from build123d import *

# Parameters (mm, degrees)
BASE_BODY_DEPTH           = 23
FORK_SLOT_19X15_REACH     = 72.915
FORK_SLOT_SKETCH_W        = 19
FORK_SLOT_SKETCH_H        = 15
CHANNEL_CUT_SKETCH_W      = 19
CHANNEL_CUT_SKETCH_H      = 40
THIN_CHANNEL_CUT_19_DEPTH = 15
LUG_SKETCH_R              = 10
LUG_WITH_BORE_DEPTH       = 10
SUPPORT_RIB_REACH         = 82.206
SUPPORT_RIB_SKETCH_WALL_W = 191.480853336
SUPPORT_RIB_SKETCH_WALL_H = 46


with BuildPart() as part:
    # Base Profile Sketch → Base Body (new, symmetric)
    with BuildSketch(Plane(origin=(0, 0, 0), x_dir=(0, 0, -1), z_dir=(1, 0, 0))):
        Polygon((-60, 0), (40, 0), (40, -15), (10, -15), (10, -30), (-30, -30), (-30, -15), (-60, -15), align=None)
    extrude(amount=BASE_BODY_DEPTH, both=True)

    # Fork Slot Sketch → Fork Slot 19x15 (cut, up to next)
    with BuildSketch(Plane(origin=(0, 0, 0), x_dir=(1, 0, 0), z_dir=(0, 1, 0)), mode=Mode.PRIVATE) as fork_slot_19x15_sk1:
        with Locations((0, -52.5)):
            Rectangle(FORK_SLOT_SKETCH_W, FORK_SLOT_SKETCH_H)
    fork_slot_19x15_tool1 = extrude(fork_slot_19x15_sk1.sketch, amount=-FORK_SLOT_19X15_REACH, mode=Mode.PRIVATE) & part.part
    add(fork_slot_19x15_tool1.solids().sort_by_distance((0, 0, 52.5))[0], mode=Mode.SUBTRACT)

    # Channel Cut Sketch → Thin Channel Cut 19 (cut)
    with BuildSketch(Plane.XZ.offset(30)):
        with Locations((0, 10)):
            Rectangle(CHANNEL_CUT_SKETCH_W, CHANNEL_CUT_SKETCH_H)
    extrude(amount=-THIN_CHANNEL_CUT_19_DEPTH, mode=Mode.SUBTRACT)

    # Lug Sketch → Lug with Bore (add)
    with BuildSketch(Plane.XY):
        with BuildLine():
            Line((23, 25), (23, 0))
            Line((23, 0), (-23, 0))
            Line((-23, 0), (-23, 25))
            ThreePointArc((-23, 25), (0, 48), (23, 25))
        make_face()
        with Locations((0, 25)):
            Circle(LUG_SKETCH_R, mode=Mode.SUBTRACT)
    extrude(amount=LUG_WITH_BORE_DEPTH)

    # Support Rib Sketch wall → Support Rib (add, up to next)
    with BuildSketch(Plane(origin=(0, 6.5, 23), x_dir=(0, -0.4472135955, 0.894427191), z_dir=(0, -0.894427191, -0.4472135955)), mode=Mode.PRIVATE) as support_rib_sk1:
        Rectangle(SUPPORT_RIB_SKETCH_WALL_W, SUPPORT_RIB_SKETCH_WALL_H)
    support_rib_tool1 = extrude(support_rib_sk1.sketch, amount=SUPPORT_RIB_REACH, mode=Mode.PRIVATE) - part.part
    add(support_rib_tool1.solids().sort_by_distance((0, 6.5, 23))[0])


solid = part.part
Can you work these out from the model? Positions are in its coordinate system, mm. A direction names the side the tool comes from. Coordinates: 2 decimals unless noted, no trailing zeros. Loops run counter-clockwise (first coordinate to the right, second up) from the corner with the lowest first, then second, coordinate; pieces in that order, holes last. Notation, with made-up numbers: (73.25, 11) - (99.25, 11) arc R25 ccw to (99.25, 40) - close; hole circle Ø3 at (-15.75, 59.5). An arc over 180 degrees is marked (long way). Put each result on its own line as item: value. Start each with the question number.
Item 1: Suppose I cut it at B-B (x = 0). Please give me the cut outline in (y, z).
Item 2: Suppose I cut it at C-C (z = -8). Please give me the cut outline in (x, y).
Item 3: For pin 1 (14 mm diameter, centred on x = 9, z = -4, fed in from -Y); pin 2 (10 mm diameter, centred on x = 0, y = 24, fed in from +Z); pin 3 (7 mm diameter, centred on x = -16, y = -23, fed in from -Z); pin 4 (7.5 mm diameter, centred on x = -1.5, y = -6.5, fed in from +Z), each with a flat end and sliding along its axis, tell me the tip position at first contact or that it passes through.
Item 4: Which directions (+Z, -Z, +X, -X, +Y, -Y) give clear straight access to the entire face, cutting with the end or side of a thin tool? Please do faces 4 (the face through (-9.5, -23, 10)), 5 (the face through (-16, -22, -10)), 6 (the face through (0, -7, 45)), 7 (the face through (-16, -23, 30)).
Item 5: If we mould it in two halves opening along Y, with no side actions, what happens to faces 1 (the face through (-1.302, 34.915, 4.93)), 2 (the face through (0, 0, -20)), 3 (the face through (9.5, -23, 10))? For each: +Y half, -Y half, draft (parallel to the pull), parting line (faces both ways), or undercut.
Item 6: If I drill on line 1 along Y through (x, z) = (0, 2.75); line 2 along Z through (x, y) = (-21, 24); line 3 along Z through (x, y) = (-2, 11.5), over which ranges is the centre line in solid material (lowest first)?
Item 7: Suppose I cut it at D-D (y = -8.5). Please give me the cut outline in (x, z).
Item 8: Suppose I cut it at A-A (y = -23). Please give me the cut outline in (x, z), and give its area (3 significant figures).
Here are the results:
1. outline: (-15, -40) - (0, -40) - (0, 0) - (15, 0) - (15, 10) - (13, 10) - (0, 36) - (0, 45) - (-15, 45) - close; (35, 0) - (48, 0) - (48, 10) - (35, 10) - close
2. outline: (-23, -30) - (-9.5, -30) - (-9.5, -15) - (9.5, -15) - (9.5, -30) - (23, -30) - (23, 0) - (-23, 0) - close
3. pin 1: y = -30
3. pin 2: through
3. pin 3: z = -10
3. pin 4: z = 45
4. face 4: +Z, -Z, -Y
4. face 5: -Z, +X, -X, -Y
4. face 6: +Z, +Y, -Y
4. face 7: +Z, +X, -X, -Y
5. face 1: undercut
5. face 2: +Y half
5. face 3: draft
6. line 1: -15 to 15, 35 to 48
6. line 2: 0 to 10
6. line 3: 0 to 13
7. outline: (-23, -40) - (23, -40) - (23, 60) - (9.5, 60) - (9.5, 45) - (-9.5, 45) - (-9.5, 60) - (-23, 60) - close
8. outline: (-23, -10) - (-9.5, -10) - (-9.5, 30) - (-23, 30) - close; (9.5, -10) - (23, -10) - (23, 30) - (9.5, 30) - close
8. area: 1,080 mm²
